For this review, take the finished solid that the model builds, in its own axes (mm). A direction names the side the tool comes from. Give positions to 0.01 mm unless a question says otherwise; leave off trailing zeros. Order: outer loops, then holes, each group sorted by start corner. A loop starts at its lowest first (then second) coordinate and runs counter-clockwise, first axis right, second up.
Item 1: Machinability: for faces 5 (the flat face through (18, 11, -17)), 6 (the cylindrical face through (-47.535, 10.676, -4.032)), 7 (the flat face through (-48, 15, 10)), 8 (the flat face through (47, 11, 0)), which of the approach directions +Z, -Z, +X, -X, +Y, -Y give a long, thin tool a straight path to every point of the face, cutting with its end or side? Answer none if there is none.
Item 2: For P1, Ø3.5, axis at x = 48, y = 17, coming from the +Z side; P2, Ø4, axis at x = 14.5, z = -17, coming from the +Y side; P3, Ø2.5, axis at x = 48.5, y = 14.5, coming from the -Z side, all flat-tipped, find the tip position at first contact; note any pin that passes through.
Item 3: Consider section D-D (x = -1). Give the boundary of the cut face in (y, z), plus the area to 3 significant figures.
Item 4: Consider section C-C (z = 6). Give the boundary of the cut face in (x, y), plus the area to 3 significant figures.
Item 5: The part is to be moulded in two halves that separate along X. For faces 1 (the flat face through (-45, 13, -7)), 2 (the flat face through (13, 11, 18)), 3 (the flat face through (50, 12, 0)), 4 (the flat face through (49, 24.132, 0)), say which applies: released by +X, released by -X, zero draft, split by the parting line, or undercut.
Item 6: For probe 1 along Y at (x, z) = (48.65, 0); probe 2 along X at (y, z) = (15, -9.5); probe 3 along Z at (x, y) = (-46.1, 17), list the stretches that pass through material, from the lowest coordinate up.
Item 7: Consider section A-A (z = 0). Give the boundary of the cut face in (x, y), plus the area to 3 significant figures.
Item 8: Consider section B-B (y = 17). Give the boundary of the cut face in (x, z), plus the area to 3 significant figures.
```python
from build123d import *

# Parameters (mm, degrees)
SKETCH1_W           = 100
SKETCH1_H           = 40
BOSS_EXTRUDE1_DEPTH = 3
SKETCH2_W           = 20
SKETCH2_H           = 25
SKETCH2_R           = 7.5
BOSS_EXTRUDE2_DEPTH = 5
SKETCH3_R           = 7.5
BOSS_EXTRUDE3_DEPTH = 5
SKETCH4_W           = 5
SKETCH4_H           = 16
BOSS_EXTRUDE4_DEPTH = 5
SKETCH7_W           = 24
SKETCH7_H           = 24.131684527
SKETCH7_R           = 4
BOSS_EXTRUDE5_DEPTH = 3
SKETCH9_W           = 8.913505449
SKETCH9_H           = 22.920442584
CUT_EXTRUDE3_DEPTH  = 47


with BuildPart() as part:
    # Sketch1 → Boss-Extrude1 (new body)
    with BuildSketch(Plane(origin=(0, 0, 0), x_dir=(1, 0, 0), z_dir=(0, 1, 0))):
        Rectangle(SKETCH1_W, SKETCH1_H)
    extrude(amount=BOSS_EXTRUDE1_DEPTH)

    # Sketch2 → Boss-Extrude2 (add)
    with BuildSketch(Plane(origin=(40, 0, 0), x_dir=(0, 0, -1), z_dir=(1, 0, 0))):
        with Locations((0, 15.5)):
            Rectangle(SKETCH2_W, SKETCH2_H)
        with Locations((0, 17)):
            Circle(SKETCH2_R, mode=Mode.SUBTRACT)
    extrude(amount=BOSS_EXTRUDE2_DEPTH)

    # Sketch3 → Boss-Extrude3 (add)
    with BuildSketch(Plane.ZY.offset(50)):
        Polygon((-10, 3), (-3.5, 3), (-3.5, 8), (3.5, 8), (3.5, 3), (10, 3), (10, 28), (-10, 28), align=None)
        with Locations(Location((0, 17, 0), (0, 0, 180))):
            Circle(SKETCH3_R, mode=Mode.SUBTRACT)
    extrude(amount=-BOSS_EXTRUDE3_DEPTH)

    # Sketch4 → Boss-Extrude4 (add)
    with BuildSketch(Plane(origin=(13, 0, 0), x_dir=(0, 0, -1), z_dir=(1, 0, 0))):
        with Locations((17.5, 11)):
            Rectangle(SKETCH4_W, SKETCH4_H)
        with Locations((-17.5, 11)):
            Rectangle(SKETCH4_W, SKETCH4_H)
    extrude(amount=BOSS_EXTRUDE4_DEPTH)

    # Sketch7 → Boss-Extrude5 (add)
    with BuildSketch(Plane(origin=(50, 0, 0), x_dir=(0, 0, -1), z_dir=(1, 0, 0))):
        with Locations((0, 12.065842264)):
            Rectangle(SKETCH7_W, SKETCH7_H)
        with Locations((0, 17)):
            Circle(SKETCH7_R, mode=Mode.SUBTRACT)
    extrude(amount=-BOSS_EXTRUDE5_DEPTH)

    # Sketch9 → Cut-Extrude3 (cut)
    with BuildSketch(Plane(origin=(0, 3, 0), x_dir=(1, 0, 0), z_dir=(0, 1, 0))):
        with Locations((40.747453483, 0)):
            Rectangle(SKETCH9_W, SKETCH9_H)
    extrude(amount=CUT_EXTRUDE3_DEPTH, mode=Mode.SUBTRACT)


solid = part.part
```
Resolved:
1. face 5: +Z, -Z, +X, +Y
1. face 6: -X
1. face 7: +Z, -X, +Y
1. face 8: +Z, -Z, +Y
2. P1: stops at z = 12
2. P2: stops at y = 19
2. P3: stops at z = -12
3. outline: (0, -20) - (3, -20) - (3, 20) - (0, 20) - close
3. area: 120 mm2
4. outline: (-50, 0) - (50, 0) - (50, 24.13) - (47, 24.13) - (47, 3) - (-45, 3) - (-45, 12.5) - (-50, 12.5) - close; (-50, 21.5) - (-45, 21.5) - (-45, 28) - (-50, 28) - close
4. area: 443 mm2
5. face 1: undercut
5. face 2: released by -X
5. face 3: released by +X
5. face 4: zero draft
6. probe 1: y = 0 to 13, 21 to 24.13
6. probe 2: x = -50 to -45, 47 to 50
6. probe 3: z = -10 to -7.5, 7.5 to 10
7. outline: (-50, 0) - (50, 0) - (50, 13) - (47, 13) - (47, 3) - (-50, 3) - close; (-50, 8) - (-45, 8) - (-45, 9.5) - (-50, 9.5) - close; (-50, 24.5) - (-45, 24.5) - (-45, 28) - (-50, 28) - close; (47, 21) - (50, 21) - (50, 24.13) - (47, 24.13) - close
7. area: 364 mm2
8. outline: (-50, -10) - (-45, -10) - (-45, -7.5) - (-50, -7.5) - close; (-50, 7.5) - (-45, 7.5) - (-45, 10) - (-50, 10) - close; (13, -20) - (18, -20) - (18, -15) - (13, -15) - close; (13, 15) - (18, 15) - (18, 20) - (13, 20) - close; (47, -12) - (50, -12) - (50, -4) - (47, -4) - close; (47, 4) - (50, 4) - (50, 12) - (47, 12) - close
8. area: 123 mm2
